Read the model definition and answer for the solid it produces. Units are mm, in the model's axes. Round coordinates to 2 decimals unless told otherwise and drop trailing zeros. Order: outer loops, then holes, each group sorted by start corner. A loop starts at its lowest first (then second) coordinate and runs counter-clockwise, first axis right, second up. Notation, with made-up numbers: (53, 77.25) - (68, 77.25) arc R29 cw to (68, 115.25) - close; hole circle Ø2 at (88.25, -16). An arc over 180 degrees is marked (long way). Put each result on its own line as item: value. Start each with the question number.
Q1. Section D-D on y = -14.5 is taken. Give the vertices of the cut face in (x, z).
Q2. Section C-C on z = 0 is taken. Give the vertices of the cut face in (x, y), then the cut area to 3 significant figures.
Q3. Find the intervals of material crossed by line 1 along Y through (x, z) = (6.5, 0); line 2 along Y through (x, z) = (4.5, 20); line 3 along Y through (x, z) = (5.5, 19), in increasing order. Write a range as from..to.
Q4. Section A-A on y = 62.5 is taken. Give the vertices of the cut face in (x, z), then the cut area to 3 significant figures.
Q5. Section B-B on z = -20 is taken. Give the vertices of the cut face in (x, y), then the cut area to 3 significant figures.
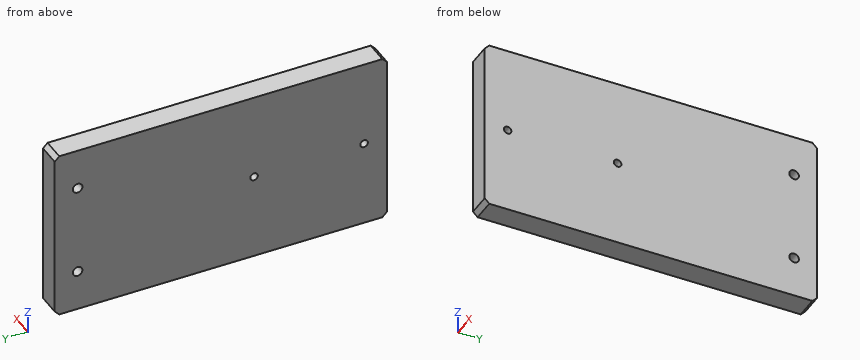
from build123d import *

# Parameters (mm, degrees)
SKETCH_1_W         = 76
SKETCH_1_H         = 145
EXTRUDE_1_DEPTH    = 10
HOLE_WIZARD_M5_1_D = 4.2
HOLE_WIZARD_M4_1_D = 3.3
CHAMFER_1_SIZE     = 2


with BuildPart() as part:
    # 草图1 → 凸台-拉伸1 (new body)
    with BuildSketch(Plane(origin=(0, 0, 0), x_dir=(0, 0, -1), z_dir=(1, 0, 0))):
        Rectangle(SKETCH_1_W, SKETCH_1_H)
    extrude(amount=EXTRUDE_1_DEPTH)

    # M5 螺纹孔1 (through all)
    with Locations(Plane.ZY):
        with Locations((20, 62.5), (-20, 62.5)):
            Hole(HOLE_WIZARD_M5_1_D / 2)

    # M4 螺纹孔1 (through all)
    with Locations(Plane.ZY):
        with Locations((0, -14.5), (0, -62.5)):
            Hole(HOLE_WIZARD_M4_1_D / 2)

    # 倒角1
    chamfer_1_edges = [part.edges().sort_by_distance(p)[0] for p in [
        (5, -72.5, -38),
        (5, -72.5, 38),
        (5, 72.5, 38),
        (5, 72.5, -38),
    ]]
    chamfer(chamfer_1_edges, length=CHAMFER_1_SIZE)


solid = part.part
Findings:
1. outline: (0, -38) - (10, -38) - (10, -1.65) - (0, -1.65) - close; (0, 1.65) - (10, 1.65) - (10, 38) - (0, 38) - close
2. outline: (0, -72.5) - (10, -72.5) - (10, -64.15) - (0, -64.15) - close; (0, -60.85) - (10, -60.85) - (10, -16.15) - (0, -16.15) - close; (0, -12.85) - (10, -12.85) - (10, 72.5) - (0, 72.5) - close
2. area: 1,380 mm2
3. line 1: -72.5..-64.15, -60.85..-16.15, -12.85..72.5
3. line 2: -72.5..60.4, 64.6..72.5
3. line 3: -72.5..60.65, 64.35..72.5
4. outline: (0, -38) - (10, -38) - (10, -22.1) - (0, -22.1) - close; (0, -17.9) - (10, -17.9) - (10, 17.9) - (0, 17.9) - close; (0, 22.1) - (10, 22.1) - (10, 38) - (0, 38) - close
4. area: 676 mm2
5. outline: (0, -72.5) - (10, -72.5) - (10, 60.4) - (0, 60.4) - close; (0, 64.6) - (10, 64.6) - (10, 72.5) - (0, 72.5) - close
5. area: 1,410 mm2
